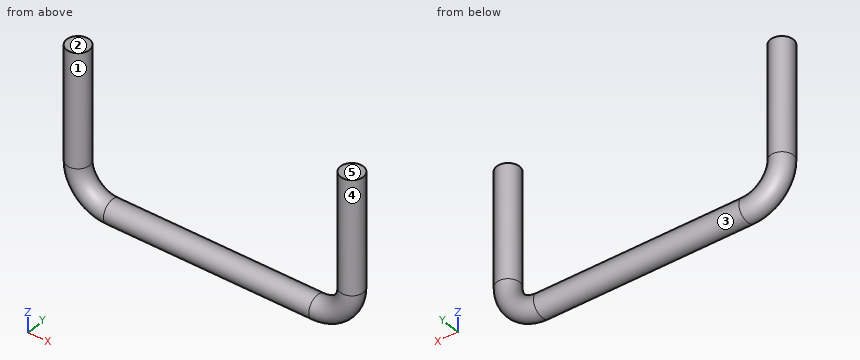
```python
from build123d import *

# Parameters (mm, degrees)
SKETCH1_R = 6.35


with BuildPart() as part:
    # Sweep1: sweep along a path in Sketch2
    with BuildLine(Plane(origin=(0, 0, 0), x_dir=(1, 0, 0), z_dir=(0, 1, 0))) as sweep1_path:
        Line((0, 0), (0, 63.5))
        ThreePointArc((0, 63.5), (5.579615818, 76.970384182), (19.05, 82.55))
        Line((19.05, 82.55), (133.35, 82.55))
        ThreePointArc((133.35, 82.55), (146.820384182, 76.970384182), (152.4, 63.5))
        Line((152.4, 63.5), (152.4, 0))
    # Sketch1 → Sweep1 (sweep)
    with BuildSketch(Plane.XY):
        Circle(SKETCH1_R)
    sweep(path=sweep1_path.line)


solid = part.part
```
The model under review builds one solid part; all positions refer to its coordinate system, in mm. Face numbers are marked on the shaded views. A direction names the side the tool comes from. Give positions to 0.01 mm unless a question says otherwise; leave off trailing zeros. Write each loop counter-clockwise with the first axis right and the second up, starting at its lowest first coordinate (ties: lowest second). Pieces come first, ordered by that corner, then holes. Notation, with made-up numbers: (28, 26.25) - (36, 26.25) arc R20 cw to (36, 30.25) - close; hole circle Ø2 at (55.5, -3). An arc over 180 degrees is marked (long way). Answer in a Markdown table with one row per item. Add a question column.
1. Tool access review of the marked faces 4 and 5: name each direction out of +Z, -Z, +X, -X, +Y, -Y from which nothing blocks a thin tool from reaching the whole face with its end or side.
2. Insertion check: P1, Ø1.5, axis at x = 75.5, y = -1, coming from the +Z side; P2, Ø12, axis at x = 14, z = -10.5, coming from the +Y side; P3, Ø6, axis at y = -3.5, z = -10.5, coming from the +X side; P4, Ø1.5, axis at x = 111.5, y = -4, coming from the -Z side. Each pin has a flat end and moves straight along its axis. Give the tip position at first contact, or say it passes through.
3. Draft analysis for pull direction X (two halves, no side actions). For the marked faces 1, 2 and 3, state which applies: +X half, -X half, draft (parallel to the pull), parting line (faces both ways), or undercut.
4. Wall thickness on line 1 along X through (y, z) = (5.5, -71); line 2 along X through (y, z) = (-0.25, -25); line 3 along Z through (x, y) = (105.5, 0): over which ranges is each line inside the solid? List them lowest first. Write a range as [from, to].
5. We need section A-A on y = 0. Write out the cut boundary in (x, z), then the cut area to 3 significant figures.
6. We need section C-C on x = 72.5. Write out the cut boundary in (y, z), then the cut area to 3 significant figures.
7. We need section B-B on z = -51. Write out the cut boundary in (x, y).
Ans:
| question | item | result |
|---|---|---|
| 1 | face 4 | +Z |
| 1 | face 5 | +Z, +X, -X, +Y, -Y |
| 2 | P1 | stops at z = -76.2 |
| 2 | P2 | passes through |
| 2 | P3 | stops at x = 158.73 |
| 2 | P4 | stops at z = -88.01 |
| 3 | face 1 | undercut |
| 3 | face 2 | draft |
| 3 | face 3 | undercut |
| 4 | line 1 | x = [-1.87, 5.06], [147.34, 154.27] |
| 4 | line 2 | x = [-6.35, 6.35], [146.05, 158.75] |
| 4 | line 3 | z = [-88.9, -76.2] |
| 5 | outline | (-6.35, -63.5) arc R25.4 ccw to (19.05, -88.9) - (133.35, -88.9) arc R25.4 ccw to (158.75, -63.5) - (158.75, 0) - (146.05, 0) - (146.05, -63.5) arc R12.7 cw to (133.35, -76.2) - (19.05, -76.2) arc R12.7 cw to (6.35, -63.5) - (6.35, 0) - (-6.35, 0) - close |
| 5 | area | 3,820 mm^2 |
| 6 | outline | circle Ø12.7 at (0, -82.55) |
| 6 | area | 127 mm^2 |
| 7 | outline | circle Ø12.7 at (0, 0); circle Ø12.7 at (152.4, 0) |
